```python
from build123d import *

# Parameters (mm, degrees)
EXTRUDE1_DEPTH = 6
SKETCH2_R      = 9
EXTRUDE2_DEPTH = 176.339670354


with BuildPart() as part:
    # Sketch1 → Extrude1 (new, symmetric)
    with BuildSketch(Plane.XY):
        with BuildLine():
            Line((80, 150), (-80, 150))
            ThreePointArc((-80, 150), (-87.071067812, 147.071067812), (-90, 140))
            Line((-90, 140), (-90, -140))
            ThreePointArc((-90, -140), (-87.071067812, -147.071067812), (-80, -150))
            Line((-80, -150), (80, -150))
            ThreePointArc((80, -150), (87.071067812, -147.071067812), (90, -140))
            Line((90, -140), (90, 140))
            ThreePointArc((90, 140), (87.071067812, 147.071067812), (80, 150))
        make_face()
    extrude(amount=EXTRUDE1_DEPTH, both=True)

    # Sketch2 → Extrude2 (cut, through all)
    with BuildSketch(Plane.XY.offset(6)):
        with Locations((-70, -130)):
            Circle(SKETCH2_R)
        with Locations((70, -130)):
            Circle(SKETCH2_R)
        with Locations((-70, 130)):
            Circle(SKETCH2_R)
        with Locations((70, 130)):
            Circle(SKETCH2_R)
    extrude(amount=-EXTRUDE2_DEPTH, mode=Mode.SUBTRACT)


solid = part.part
```
CAD build for the part. Positions are in the model's coordinates, mm. Round coordinates to 2 decimals unless told otherwise and drop trailing zeros. Loops run counter-clockwise (first coordinate to the right, second up) from the corner with the lowest first, then second, coordinate; pieces in that order, holes last. Notation, with made-up numbers: M -11,4 L 32,4 A21 ccw 32,31 Z; hole C 42.25,73.5 d10. An arc over 180 degrees is marked long. Return JSON: item names as keys, results as strings. Group by question number.
(1) Saw through at B-B, the plane x = 70. List the corners of the cut face in (y, z), and give its area (3 significant figures).
(2) Saw through at C-C, the plane z = -3.75. List the corners of the cut face in (x, y).
(3) Saw through at A-A, the plane y = -130. List the corners of the cut face in (x, z), and give its area (3 significant figures).
(4) Mould opens along Y. For faces 1 (the cylindrical face through (-65.16, -122.41, 0.08)), 2 (the flat face through (-1, 2, 6)), 3 (the cylindrical face through (-65.16, 137.59, 0.08)), 4 (the cylindrical face through (86.99, -147.15, 0.08)) say: +Y half, -Y half, draft (parallel to the pull), parting line (faces both ways), or undercut.
(5) Wall check: probe 1 along X at (y, z) = (-131, -0.75); probe 2 along Y at (x, z) = (-70, 2); probe 3 along Y at (x, z) = (62, 0.75). Give the ranges that are in metal, low to high. Write a range as [from, to].
Answer list:
{
 "1": {"outline": "M -150,-6 L -139,-6 L -139,6 L -150,6 Z; M -121,-6 L 121,-6 L 121,6 L -121,6 Z; M 139,-6 L 150,-6 L 150,6 L 139,6 Z", "area": "3,170 mm2"},
 "2": {"outline": "M -90,-140 A10 ccw -80,-150 L 80,-150 A10 ccw 90,-140 L 90,140 A10 ccw 80,150 L -80,150 A10 ccw -90,140 Z; hole C -70,-130 d18; hole C -70,130 d18; hole C 70,-130 d18; hole C 70,130 d18"},
 "3": {"outline": "M -90,-6 L -79,-6 L -79,6 L -90,6 Z; M -61,-6 L 61,-6 L 61,6 L -61,6 Z; M 79,-6 L 90,-6 L 90,6 L 79,6 Z", "area": "1,730 mm2"},
 "4": {"face 1": "undercut", "face 2": "draft", "face 3": "undercut", "face 4": "-Y half"},
 "5": {"probe 1": "[-90, -78.94], [-61.06, 61.06], [78.94, 90]", "probe 2": "[-150, -139], [-121, 121], [139, 150]", "probe 3": "[-150, -134.12], [-125.88, 125.88], [134.12, 150]"}
}
